```python
from build123d import *

# Parameters (mm, degrees)
HOUSING_PROFILE_SKETCH_R      = 52.5
HOUSING_PROFILE_SKETCH_R_2    = 40.5
BEARING_HOUSING_BOSS_DEPTH    = 63
MOUNTING_FLANGE_12MM_DEPTH    = 12
SKETCH1_4_R                   = 23.666666665
SKETCH1_4_R_2                 = 11.666666665
BOLT_LUG_BOSSES_25MM_DEPTH    = 25
FLANGE_POCKETS_3MM_DEEP_DEPTH = 3


with BuildPart() as part:
    # Housing Profile Sketch → Bearing Housing Boss (new body)
    with BuildSketch(Plane(origin=(0, 0, 0), x_dir=(1, 0, 0), z_dir=(0, 1, 0))):
        with Locations(Location((0, 0, 0), (0, 0, 270))):
            Circle(HOUSING_PROFILE_SKETCH_R)
        with Locations(Location((0, 0, 0), (0, 0, 270))):
            Circle(HOUSING_PROFILE_SKETCH_R_2, mode=Mode.SUBTRACT)
    extrude(amount=BEARING_HOUSING_BOSS_DEPTH)

    # Sketch1_3 → Mounting Flange 12mm (add)
    with BuildSketch(Plane(origin=(0, 0, 0), x_dir=(1, 0, 0), z_dir=(0, 1, 0))):
        with BuildLine():
            ThreePointArc((-17.300000001, -49.567731439), (-52.5, 0), (-17.300000001, 49.567731439))
            Line((-17.300000001, 49.567731439), (-95.298730159, 22.344818615))
            ThreePointArc((-95.298730159, 22.344818615), (-73.797059367, 19.296127307), (-63.833333335, 0))
            ThreePointArc((-63.833333335, 0), (-73.797059367, -19.296127307), (-95.298730159, -22.344818615))
            Line((-95.298730159, -22.344818615), (-17.300000001, -49.567731439))
        make_face()
        with BuildLine():
            Line((95.298730159, 22.344818615), (17.300000001, 49.567731439))
            ThreePointArc((17.300000001, 49.567731439), (42.804789452, 30.397368307), (52.5, 0))
            ThreePointArc((52.5, 0), (42.804789452, -30.397368307), (17.300000001, -49.567731439))
            Line((17.300000001, -49.567731439), (95.298730159, -22.344818615))
            ThreePointArc((95.298730159, -22.344818615), (63.833333335, 0), (95.298730159, 22.344818615))
        make_face()
    extrude(amount=MOUNTING_FLANGE_12MM_DEPTH)

    # Sketch1_4 → Bolt Lug Bosses 25mm (add)
    # profile 1 of 2: a face of its own
    with BuildSketch(Plane(origin=(0, 0, 0), x_dir=(1, 0, 0), z_dir=(0, 1, 0))):
        with Locations(Location((-87.5, 0, 0), (0, 0, 109.239875226))):
            Circle(SKETCH1_4_R)
        with Locations(Location((-87.5, 0, 0), (0, 0, 270))):
            Circle(SKETCH1_4_R_2, mode=Mode.SUBTRACT)
    # profile 2 of 2: a face of its own
    with BuildSketch(Plane(origin=(0, 0, 0), x_dir=(1, 0, 0), z_dir=(0, 1, 0))):
        with Locations(Location((87.5, 0, 0), (0, 0, 70.760124774))):
            Circle(SKETCH1_4_R)
        with Locations(Location((87.5, 0, 0), (0, 0, 270))):
            Circle(SKETCH1_4_R_2, mode=Mode.SUBTRACT)
    extrude(amount=BOLT_LUG_BOSSES_25MM_DEPTH)

    # Flange Pocket Sketch → Flange Pockets 3mm Deep (cut)
    with BuildSketch(Plane(origin=(0, 12, 0), x_dir=(1, 0, 0), z_dir=(0, 1, 0))):
        with BuildLine():
            Line((-40.009336858, 38.464307665), (-77.89822284, 25.240427764))
            ThreePointArc((-77.89822284, 25.240427764), (-60.494939024, 0), (-77.89822284, -25.240427764))
            Line((-77.89822284, -25.240427764), (-40.009336858, -38.464307665))
            ThreePointArc((-40.009336858, -38.464307665), (-55.5, 0), (-40.009336858, 38.464307665))
        make_face()
        with BuildLine():
            Line((40.009336858, 38.464307665), (77.732740957, 25.298183818))
            ThreePointArc((77.732740957, 25.298183818), (60.381787417, 0), (77.732740957, -25.298183818))
            Line((77.732740957, -25.298183818), (40.009336858, -38.464307665))
            ThreePointArc((40.009336858, -38.464307665), (55.5, 0), (40.009336858, 38.464307665))
        make_face()
    extrude(amount=-FLANGE_POCKETS_3MM_DEEP_DEPTH, mode=Mode.SUBTRACT)


solid = part.part
```
Geometry: final body of the model. Coordinates: model frame, mm. A direction names the side the tool comes from. Give positions to 0.01 mm unless a question says otherwise; leave off trailing zeros. Loops run counter-clockwise (first coordinate to the right, second up) from the corner with the lowest first, then second, coordinate; pieces in that order, holes last. Notation, with made-up numbers: (58.5, 6) -> (112.5, 6) arc R16 cw to (112.5, 33) -> close; hole circle Ø10 at (46.5, 33.25). An arc over 180 degrees is marked (long way). Use one line per item in the form item = value.
Item 1: Section query B-B on y = 15.5. Output: boundary loops of the cut face in (x, z).
A:
outline = circle Ø47.33 at (-87.5, 0); circle Ø105 at (0, 0); circle Ø47.33 at (87.5, 0); hole circle Ø23.33 at (-87.5, 0); hole circle Ø81 at (0, 0); hole circle Ø23.33 at (87.5, 0)
Item 2: Pin query (flat end, axial travel): P1, Ø11.5, axis at x = -62, z = 5, coming from the +Y side; P2, Ø10, axis at y = 6.5, z = 10.5, coming from the -X side; P3, Ø4, axis at x = -26, y = 44, coming from the -Z side. Return the tip coordinate at first contact, or that it passes through.
A:
P1 = 25
P2 = -110.52
P3 = -46.69
Item 3: Access query for faces 1 (the face through (34.15, 31.06, 21.77)), 2 (the face through (-110.534, 15.103, -5.437)). Directions: +Z, -Z, +X, -X, +Y, -Y. A direction counts if a zero-diameter tool reaches every point of the face in a straight line with its end or side. Return the directions, or none.
A:
face_1 = +Y, -Y
face_2 = +Y
Item 4: Section query D-D on z = -33.5. Output: boundary loops of the cut face in (x, y).
A:
outline = (-63.34, 0) -> (-22.76, 0) -> (-22.76, 63) -> (-40.42, 63) -> (-40.42, 12) -> (-44.25, 12) -> (-44.25, 9) -> (-54.23, 9) -> (-54.23, 12) -> (-63.34, 12) -> close; (22.76, 0) -> (63.34, 0) -> (63.34, 12) -> (54.23, 12) -> (54.23, 9) -> (44.25, 9) -> (44.25, 12) -> (40.42, 12) -> (40.42, 63) -> (22.76, 63) -> close
Item 5: Section query C-C on z = 0. Give the number of separate pieces and of enclosed holes in the cut face, and give its area (3 significant figures).
A:
separate_pieces = 4
enclosed_holes = 0
area = 2,950 mm^2
Item 6: Line query: probe 1 along X at (y, z) = (23, 0); probe 2 along X at (y, z) = (22, 19); probe 3 along Z at (x, y) = (87, 11). Output: solid intervals per line, ascending.
A:
probe_1 = -111.17 to -99.17, -75.83 to -63.83, -52.5 to -40.5, 40.5 to 52.5, 63.83 to 75.83, 99.17 to 111.17
probe_2 = -101.61 to -73.39, -48.94 to -35.77, 35.77 to 48.94, 73.39 to 101.61
probe_3 = -25.24 to -11.66, 11.66 to 25.24
Item 7: Section query A-A on x = 0. Output: boundary loops of the cut face in (y, z), and give its area (3 significant figures).
A:
outline = (0, -52.5) -> (63, -52.5) -> (63, -40.5) -> (0, -40.5) -> close; (0, 40.5) -> (63, 40.5) -> (63, 52.5) -> (0, 52.5) -> close
area = 1,510 mm^2
Item 8: Draft query along X for faces 3 (the face through (56.845, 5.916, -35.766)), 4 (the face through (59, 9, 3)), 5 (the face through (-99.4, 25, -1.1)). Return one class per face: pulls with the +X half, pulls with the -X half, needs draft (parallel to the pull), parting line crosses it, or undercut.
A:
face_3 = pulls with the +X half
face_4 = undercut
face_5 = needs draft
